The listing builds one solid part. Answer for the finished solid, in the listing's coordinates (mm). A direction names the side the tool comes from. Give positions to 0.01 mm unless a question says otherwise; leave off trailing zeros. Write each loop counter-clockwise with the first axis right and the second up, starting at its lowest first coordinate (ties: lowest second). Pieces come first, ordered by that corner, then holes. Notation, with made-up numbers: (59.25, -14) - (77.25, -14) arc R28 cw to (77.25, 25) - close; hole circle Ø6 at (11.25, 86). An arc over 180 degrees is marked (long way). Use a Markdown table: item, result. Add a question column.
from build123d import *

# Parameters (mm, degrees)
SKETCH_1_R          = 2.85
EXTRUDE_1_DEPTH     = 3
CUT_EXTRUDE_1_DEPTH = 4
CHAMFER_1_SIZE      = 0.2
SKETCH_3_R          = 1.5
EXTRUDE_2_DEPTH     = 6


with BuildPart() as part:
    # 草图1 → 凸台-拉伸1 (new body)
    with BuildSketch(Plane.XY):
        Circle(SKETCH_1_R)
    extrude(amount=EXTRUDE_1_DEPTH)

    # 草图2 → 切除-拉伸1 (cut)
    with BuildSketch(Plane.XY.offset(3)):
        Polygon((0, 1.443375673), (-1.25, 0.721687836), (-1.25, -0.721687836), (0, -1.443375673), (1.25, -0.721687836), (1.25, 0.721687836), align=None)
    extrude(amount=-CUT_EXTRUDE_1_DEPTH, mode=Mode.SUBTRACT)

    # 倒角1
    chamfer_1_edges = [part.edges().sort_by_distance(p)[0] for p in [
        (-2.85, 0, 3),
    ]]
    chamfer(chamfer_1_edges, length=CHAMFER_1_SIZE)

    # 草图3 → 凸台-拉伸2 (add)
    with BuildSketch(Plane(origin=(0, 0, 0), x_dir=(-1, 0, 0), z_dir=(0, 0, -1))):
        with Locations(Location((0, 0, 0), (0, 0, 180))):
            Circle(SKETCH_3_R)
    extrude(amount=EXTRUDE_2_DEPTH)


solid = part.part
1. Given P1, Ø0.8, axis at x = -0.5, y = -0.5, coming from the +Z side; P2, Ø1.5, axis at x = 1.5, z = 0.5, coming from the +Y side; P3, Ø0.7, axis at y = 0.5, z = 1, coming from the +X side; P4, Ø1, axis at y = 0.5, z = 0.5, coming from the -X side, each flat-ended and moving along its own axis, determine where each tip first touches the part or whether it passes through.
2. The part is cut by section B-B (y = 0). Give the vertices of the cut face in (x, z).
3. Consider L1, parallel to Z at x = -1.05, y = -0.3; L2, parallel to Z at x = -2.05, y = 1.35; L3, parallel to X at y = 0.25, z = 1.25. Determine where each line is inside the solid, lowest interval first. Write a range as [from, to].
4. The part is cut by section A-A (z = 1). Give the vertices of the cut face in (x, y).
5. For a pull along Y with two mould halves and no side action, classify faces 1 (the cylindrical face through (1.43, -0.45, -2.96)), 2 (the flat face through (1.1, -1.1, 3)), 3 (the flat face through (-1.25, 0, 2)) as released by +Y, released by -Y, zero draft, split by the parting line, or undercut.
6. Which of the six approach directions +Z, -Z, +X, -X, +Y, -Y give full straight-line access (tool end or side, diameter ignored) to faces 4 (the flat face through (-0.63, -1.08, 1.52)), 5 (the flat face through (0, 0, -6)), 6 (the flat face through (1.2, -1.2, 0))?
Check values:
| question | item | result |
|---|---|---|
| 1 | P1 | stops at z = 0 |
| 1 | P2 | stops at y = 2.75 |
| 1 | P3 | stops at x = 2.85 |
| 1 | P4 | stops at x = -2.85 |
| 2 | outline | (-2.85, 0) - (-1.5, 0) - (-1.5, -6) - (1.5, -6) - (1.5, 0) - (2.85, 0) - (2.85, 2.8) - (2.65, 3) - (1.25, 3) - (1.25, 0) - (-1.25, 0) - (-1.25, 3) - (-2.65, 3) - (-2.85, 2.8) - close |
| 3 | L1 | z = [-6, 0] |
| 3 | L2 | z = [0, 3] |
| 3 | L3 | x = [-2.84, -1.25], [1.25, 2.84] |
| 4 | outline | circle Ø5.7 at (0, 0); hole (-1.25, -0.72) - (0, -1.44) - (1.25, -0.72) - (1.25, 0.72) - (0, 1.44) - (-1.25, 0.72) - close |
| 5 | face 1 | split by the parting line |
| 5 | face 2 | zero draft |
| 5 | face 3 | undercut |
| 6 | face 4 | +Z |
| 6 | face 5 | -Z, +X, -X, +Y, -Y |
| 6 | face 6 | -Z |
